Verification items for the finished model (mm, model axes). Give positions to 0.01 mm unless a question says otherwise; leave off trailing zeros. Loops run counter-clockwise (first coordinate to the right, second up) from the corner with the lowest first, then second, coordinate; pieces in that order, holes last. Notation, with made-up numbers: (1, 57) - (59, 57) arc R21 ccw to (59, 63) - close; hole circle Ø5 at (-24.75, -5). An arc over 180 degrees is marked (long way). Answer in a Markdown table with one row per item.
```python
from build123d import *

# Parameters (mm, degrees)
SKETCH_1_R             = 20
EXTRUDE_1_DEPTH        = 1635.36
SKETCH_2_R             = 15
EXTRUDE_2_DEPTH        = 35
EXTRUDE_START          = 35
SKETCH_3_R             = 15
EXTRUDE_3_DEPTH        = 35
CUT_EXTRUDE_1_DEPTH    = 1671.846351284
SKETCH_5_W             = 1.85
SKETCH_5_H             = 1.25
SKETCH_7_W             = 1.85
SKETCH_7_H             = 1.25
PATTERN_LINEAR_2_COUNT = 2
PATTERN_LINEAR_2_PITCH = 60


with BuildPart() as part:
    # 草图1 → 凸台-拉伸1 (new body)
    with BuildSketch(Plane(origin=(0, 0, 0), x_dir=(0, 0, -1), z_dir=(1, 0, 0))):
        Circle(SKETCH_1_R)
    extrude(amount=EXTRUDE_1_DEPTH)

    # 草图2 → 凸台-拉伸2 (add)
    with BuildSketch(Plane.ZY):
        Circle(SKETCH_2_R)
    extrude(amount=EXTRUDE_2_DEPTH)

    # 草图3 → 凸台-拉伸3 (add)
    with BuildSketch(Plane(origin=(1635.36, 0, 0), x_dir=(0, 0, -1), z_dir=(1, 0, 0)).offset(EXTRUDE_START)):
        with Locations(Location((0, 0, 0), (0, 0, 180))):
            Circle(SKETCH_3_R)
    extrude(amount=-EXTRUDE_3_DEPTH)

    # 草图4 → 切除-拉伸1 (cut, through all)
    with BuildSketch(Plane.XY.offset(15)):
        with BuildLine():
            Line((13.3, 6), (28.3, 6))
            ThreePointArc((28.3, 6), (34.3, 0), (28.3, -6))
            Line((28.3, -6), (13.3, -6))
            ThreePointArc((13.3, -6), (7.3, 0), (13.3, 6))
        make_face()
        with BuildLine():
            Line((1622.06, -6), (1607.06, -6))
            ThreePointArc((1607.06, -6), (1601.06, 0), (1607.06, 6))
            Line((1607.06, 6), (1622.06, 6))
            ThreePointArc((1622.06, 6), (1628.06, 0), (1622.06, -6))
        make_face()
        with BuildLine():
            Line((1562.06, -6), (1547.06, -6))
            ThreePointArc((1547.06, -6), (1541.06, 0), (1547.06, 6))
            Line((1547.06, 6), (1562.06, 6))
            ThreePointArc((1562.06, 6), (1568.06, 0), (1562.06, -6))
        make_face()
    extrude(amount=CUT_EXTRUDE_1_DEPTH, mode=Mode.SUBTRACT)

    # 草图5 → 切除-旋转1 (revolve, cut)
    with BuildSketch(Plane.XY, mode=Mode.PRIVATE) as cut_revolve_1_sk:
        with Locations((4.875, 19.375)):
            Rectangle(SKETCH_5_W, SKETCH_5_H)
        with Locations((36.725, 19.375)):
            Rectangle(SKETCH_5_W, SKETCH_5_H)
    revolve(cut_revolve_1_sk.sketch.rotate(Axis((0, 0, 0), (1, 0, 0)), 90), axis=Axis((0, 0, 0), (1, 0, 0)), mode=Mode.SUBTRACT)

    # 草图7 → 切除-旋转2 (revolve, cut)
    with BuildSketch(Plane.XY, mode=Mode.PRIVATE) as cut_revolve_2_sk:
        with Locations((1598.635, 19.375)):
            Rectangle(SKETCH_7_W, SKETCH_7_H)
        with Locations((1630.485, 19.375)):
            Rectangle(SKETCH_7_W, SKETCH_7_H)
    cut_revolve_2 = revolve(cut_revolve_2_sk.sketch.rotate(Axis((1670.36, 0, 0), (-1, 0, 0)), 270), axis=Axis((1670.36, 0, 0), (-1, 0, 0)), mode=Mode.SUBTRACT)

    # 阵列(线性)2: 切除-旋转2 ×2
    with Locations(*[(-i * PATTERN_LINEAR_2_PITCH, 0, 0) for i in range(1, PATTERN_LINEAR_2_COUNT)]):
        add(cut_revolve_2, mode=Mode.SUBTRACT)


solid = part.part
```
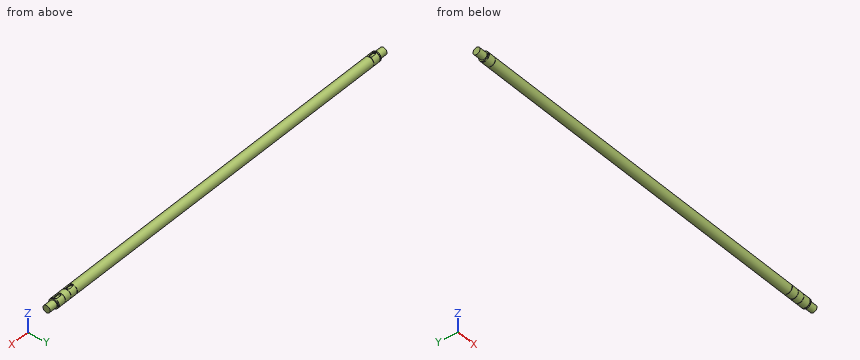
Q1. Go/stop test with flat-tipped pins: P1, Ø6, axis at x = 535.5, z = -4, coming from the -Y side (3 decimals); P2, Ø8, axis at x = 739.5, z = -9, coming from the -Y side; P3, Ø3, axis at x = 968.5, z = -12.5, coming from the -Y side. Record where each tip stops, or that it passes through.
Completed:
| item | result |
|---|---|
| P1 | y = -19.975 |
| P2 | y = -19.36 |
| P3 | y = -16.7 |
Q2. Sectioned sample at A-A (x = 388.5). Record the cut outline in (y, z), and give its area (3 significant figures).
Completed:
| item | result |
|---|---|
| outline | circle Ø40 at (0, 0) |
| area | 1,260 mm^2 |
Q3. Thickness scan on line 1 (Y direction, x = 995, z = -0.5); line 2 (Y direction, x = 778, z = 13); line 3 (Z direction, x = 171.5, y = 6). Record the ranges inside material, lowest first.
Completed:
| item | result |
|---|---|
| line 1 | -19.99 to 19.99 |
| line 2 | -15.2 to 15.2 |
| line 3 | -19.08 to 19.08 |
